Could you check a few things on this model? Use its own coordinates, in mm. A direction names the side the tool comes from. Coordinates: 2 decimals unless noted, no trailing zeros. Write each loop counter-clockwise with the first axis right and the second up, starting at its lowest first coordinate (ties: lowest second). Pieces come first, ordered by that corner, then holes. Notation, with made-up numbers: (39.5, 65) - (48.5, 65) arc R21 ccw to (48.5, 99) - close; hole circle Ø11 at (68.5, 65.25). An arc over 180 degrees is marked (long way). Answer as a JSON object with one key per item and string values. Group by question number.
1) If we section it at A-A (x = 143.5): Write out the boundary of the cut face in (y, z), plus the area to 3 significant figures.
2) On a 3-axis mill with a long thin cutter (end or side, diameter ignored), from which of +Z, -Z, +X, -X, +Y, -Y can I reach the whole of each face in a straight line? I mean faces 1 (the cylindrical face through (161.126, 2.681, 6.466)), 2 (the cylindrical face through (1.19, -6.76, -21.46)), 3 (the cylindrical face through (162, 0, 24)), 4 (the cylindrical face through (-162, 0, 24)), 5 (the cylindrical face through (-68, 0, 24)). Say none if no direction works.
3) We'd pull the mould along Z, two halves only. Please class faces 6 (the cylindrical face through (-87.465, 15.516, 20.236)), 7 (the flat face through (90, 23, 0)), 8 (the conical face through (-148.524, 1.187, -0.264)): released by +Z, released by -Z, zero draft, split by the parting line, or undercut.
4) Please list where these lines run through material, in increasing order: line 1 along Y through (x, z) = (165, 0); line 2 along X through (y, z) = (-20, -14); line 3 along Y through (x, z) = (117.5, 10.5).
5) If we section it at B-B (x = -95): Write out the boundary of the cut face in (y, z), plus the area to 3 significant figures.
6) Will these pins go through, and if not, where does the flat tip stop? pin 1 Ø1.4 at (x, z) = (48, 25) entering from +Y; pin 2 Ø3 at (x, z) = (-105.5, -12) entering from -Y; pin 3 Ø2.5 at (x, z) = (-139.5, 23) entering from -Y.
```python
from build123d import *

# Parameters (mm, degrees)
CHAMFER1_SIZE        = 1
BOSS_EXTRUDE1_DEPTH  = 26
MIRROR6_COPY_1_DEPTH = 26


with BuildPart() as part:
    # Sketch1 → Revolve1 (revolve)
    with BuildSketch(Plane.XY, mode=Mode.PRIVATE) as revolve1_sk:
        Polygon((170, 0), (-170, 0), (-170, 22.5), (-90, 22.5), (-90, 25.5), (-85, 25.5), (-85, 22.5), (85, 22.5), (85, 25.5), (90, 25.5), (90, 22.5), (170, 22.5), align=None)
    revolve(revolve1_sk.sketch.rotate(Axis((170, 0, 0), (-1, 0, 0)), 90), axis=Axis((170, 0, 0), (-1, 0, 0)))

    # Chamfer1
    chamfer1_edges = [part.edges().sort_by_distance(p)[0] for p in [
        (-170, 0, 22.5),
        (170, 0, 22.5),
    ]]
    chamfer(chamfer1_edges, length=CHAMFER1_SIZE)

    # Sketch2 → Boss-Extrude1 (add)
    with BuildSketch(Plane.XY):
        with BuildLine():
            Line((-155, 7), (-109, 7))
            ThreePointArc((-109, 7), (-102, 0), (-109, -7))
            Line((-109, -7), (-155, -7))
            ThreePointArc((-155, -7), (-162, 0), (-155, 7))
        make_face()
    boss_extrude1 = extrude(amount=BOSS_EXTRUDE1_DEPTH)

    # Mirror1: Boss-Extrude1 across plane
    add(boss_extrude1.mirror(Plane(origin=(0, 0, 0), x_dir=(0, 0, 1), z_dir=(1, 0, 0))))

    # Sketch3 → M16 Tapped Hole1 (revolve, cut)
    with BuildSketch(Plane(origin=(-170, 0, 0), x_dir=(0, 0, 1), z_dir=(0, 1, 0))):
        Polygon((0, 0), (0, 22.206024333), (7, 18), (7, 0), align=None)
    m16_tapped_hole1 = revolve(axis=Axis((-176.35, 0, 0), (1, 0, 0)), mode=Mode.SUBTRACT)

    # Mirror2: M16 Tapped Hole1 across plane
    add(m16_tapped_hole1.mirror(Plane(origin=(0, 0, 0), x_dir=(0, 0, 1), z_dir=(1, 0, 0))), mode=Mode.SUBTRACT)

    # Mirror3: Boss-Extrude1 across plane
    add(boss_extrude1.mirror(Plane(origin=(-85, 25.5, 0), x_dir=(0, 0, 1), z_dir=(1, 0, 0))))

    # Mirror6 copy 1 sketch → Mirror6 copy 1 (add)
    with BuildSketch(Plane(origin=(170, 0, 0), x_dir=(1, 0, 0), z_dir=(0, 0, 1))):
        with BuildLine():
            Line((-155, 7), (-109, 7))
            ThreePointArc((-109, 7), (-102, 0), (-109, -7))
            Line((-109, -7), (-155, -7))
            ThreePointArc((-155, -7), (-162, 0), (-155, 7))
        make_face()
    extrude(amount=MIRROR6_COPY_1_DEPTH)


solid = part.part
```
Here are the results:
{
 "1": {"outline": "(-7, 21.38) arc R22.5 ccw (long way) to (7, 21.38) - (7, 26) - (-7, 26) - close", "area": "1,640 mm²"},
 "2": {"face 1": "+X", "face 2": "none", "face 3": "+Z, +X", "face 4": "+Z, -X", "face 5": "+Z"},
 "3": {"face 6": "split by the parting line", "face 7": "zero draft", "face 8": "undercut"},
 "4": {"line 1": "y = -22.5 to -7, 7 to 22.5", "line 2": "x = -90 to -85, 85 to 90", "line 3": "y = -19.9 to 19.9"},
 "5": {"outline": "circle Ø45 at (0, 0)", "area": "1,590 mm²"},
 "6": {"pin 1": "stops at y = 7", "pin 2": "stops at y = -19.9", "pin 3": "stops at y = -7"}
}
